```python
from build123d import *

# Parameters (mm, degrees)
SKETCH_2_W             = 85
SKETCH_2_H             = 230
EXTRUDE_1_DEPTH        = 12
CUT_EXTRUDE_2_DEPTH    = 2
HOLE_WIZARD_M5_1_D     = 4.2
HOLE_WIZARD_M4_1_D     = 3.3
HOLE_WIZARD_M6_1_D     = 5
HOLE_WIZARD_M6_1_DEPTH = 15
HOLE_WIZARD_M6_1_TIP   = 1.502151548
CHAMFER_1_SIZE         = 2


with BuildPart() as part:
    # 草图2 → 凸台-拉伸1 (new body)
    with BuildSketch(Plane.XY):
        Rectangle(SKETCH_2_W, SKETCH_2_H)
    extrude(amount=EXTRUDE_1_DEPTH)

    # 草图16 → 切除-拉伸2 (cut)
    with BuildSketch(Plane.XY.offset(12)):
        with BuildLine():
            Line((-22, 110), (22, 110))
            ThreePointArc((22, 110), (24.121320344, 109.121320344), (25, 107))
            Line((25, 107), (25, 53))
            ThreePointArc((25, 53), (24.121320344, 50.878679656), (22, 50))
            Line((22, 50), (-22, 50))
            ThreePointArc((-22, 50), (-24.121320344, 50.878679656), (-25, 53))
            Line((-25, 53), (-25, 107))
            ThreePointArc((-25, 107), (-24.121320344, 109.121320344), (-22, 110))
        make_face()
        with BuildLine():
            Line((-37.5, -115), (37.5, -115))
            Line((37.5, -115), (37.5, -48))
            ThreePointArc((37.5, -48), (36.621320344, -45.878679656), (34.5, -45))
            Line((34.5, -45), (-34.5, -45))
            ThreePointArc((-34.5, -45), (-36.621320344, -45.878679656), (-37.5, -48))
            Line((-37.5, -48), (-37.5, -115))
        make_face()
    extrude(amount=-CUT_EXTRUDE_2_DEPTH, mode=Mode.SUBTRACT)

    # M5 螺纹孔1 (through all)
    with Locations(Plane(origin=(0, 0, 0), x_dir=(-1, 0, 0), z_dir=(0, 0, -1))):
        with Locations((-17.5, -75), (17.5, -75), (17.5, -105), (-17.5, -105)):
            Hole(HOLE_WIZARD_M5_1_D / 2)

    # M4 螺纹孔1 (through all)
    with Locations(Plane.XY.offset(12)):
        with Locations((-20, 69), (20, 69), (-20, 91), (20, 91)):
            Hole(HOLE_WIZARD_M4_1_D / 2)

    # M6 螺纹孔1
    with Locations(Plane(origin=(0, 0, 0), x_dir=(-1, 0, 0), z_dir=(0, 0, -1))):
        with Locations((-35, 107.5), (-35, 69.5), (35, 69.5), (35, 107.5), (-35, 7.5), (-35, -30.5), (35, -30.5), (35, 7.5)):
            Hole(HOLE_WIZARD_M6_1_D / 2, depth=HOLE_WIZARD_M6_1_DEPTH)
            with Locations((0, 0, -(HOLE_WIZARD_M6_1_DEPTH + HOLE_WIZARD_M6_1_TIP / 2))):  # 118° drill point
                Cone(0, HOLE_WIZARD_M6_1_D / 2, HOLE_WIZARD_M6_1_TIP, mode=Mode.SUBTRACT)

    # 倒角1
    chamfer_1_edges = [part.edges().sort_by_distance(p)[0] for p in [
        (42.5, -115, 6),
        (-42.5, -115, 6),
        (-42.5, 115, 6),
        (42.5, 115, 6),
    ]]
    chamfer(chamfer_1_edges, length=CHAMFER_1_SIZE)


solid = part.part
```
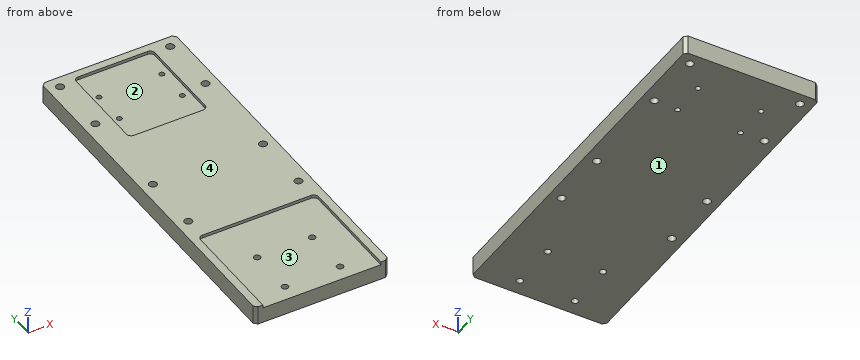
CAD build for the part. Positions are in the model's coordinates, mm. Face numbers are marked on the shaded views. A direction names the side the tool comes from. Coordinates: 2 decimals unless noted, no trailing zeros. Order: outer loops, then holes, each group sorted by start corner. A loop starts at its lowest first (then second) coordinate and runs counter-clockwise, first axis right, second up. Notation, with made-up numbers: (15.5, 23) - (38.5, 23) arc R15 ccw to (38.5, 42) - close; hole circle Ø1 at (-20.75, 0). An arc over 180 degrees is marked (long way). Answer in a Markdown table with one row per item.
1. Slice it at C-C, the plane x = -3.5. List the corners of the cut face in (y, z).
Answer:
| item | result |
|---|---|
| outline | (-115, 0) - (115, 0) - (115, 12) - (110, 12) - (110, 10) - (50, 10) - (50, 12) - (-45, 12) - (-45, 10) - (-115, 10) - close |
2. 3-axis set-ups, long thin cutter, end or side, ignore diameter. For the marked faces 3 and 4: which of +Z, -Z, +X, -X, +Y, -Y reach the whole face in a straight line?
Answer:
| item | result |
|---|---|
| face 3 | +Z, -Y |
| face 4 | +Z, +X, -X, +Y, -Y |
3. Slice it at A-A, the plane y = 7.5. List the corners of the cut face in (x, z), then the cut area to 3 significant figures.
Answer:
| item | result |
|---|---|
| outline | (-42.5, 0) - (-37.5, 0) - (-37.5, 12) - (-42.5, 12) - close; (-32.5, 0) - (32.5, 0) - (32.5, 12) - (-32.5, 12) - close; (37.5, 0) - (42.5, 0) - (42.5, 12) - (37.5, 12) - close |
| area | 900 mm² |
4. Drill centre lines: L1, parallel to Y at x = -35, z = 3.5; L2, parallel to X at y = 91, z = 5.75; L3, parallel to Y at x = 20, z = 6. Where is each one in solid material? Low to high. Write a range as from..to.
Answer:
| item | result |
|---|---|
| L1 | -115..-33, -28..5, 10..67, 72..105, 110..115 |
| L2 | -42.5..-21.65, -18.35..18.35, 21.65..42.5 |
| L3 | -115..67.35, 70.65..89.35, 92.65..115 |
5. Pull direction Y, two halves, no side cores. Call the marked faces 1 and 2: +Y half, -Y half, draft (parallel to the pull), parting line (faces both ways), or undercut.
Answer:
| item | result |
|---|---|
| face 1 | draft |
| face 2 | undercut |
6. Flat gauge pins, fed straight in: P1, Ø6.5, axis at x = -17.5, y = -75, coming from the -Z side; P2, Ø1.6, axis at x = -7.5, z = 11.5, coming from the -Y side; P3, Ø5.5, axis at x = 20, y = 91, coming from the +Z side. Where does each tip first touch, or does it go through?
Answer:
| item | result |
|---|---|
| P1 | z = 0 |
| P2 | y = -45 |
| P3 | z = 10 |
7. Slice it at D-D, the plane y = 81.5. List the corners of the cut face in (x, z), then the cut area to 3 significant figures.
Answer:
| item | result |
|---|---|
| outline | (-42.5, 0) - (42.5, 0) - (42.5, 12) - (25, 12) - (25, 10) - (-25, 10) - (-25, 12) - (-42.5, 12) - close |
| area | 920 mm² |
8. Slice it at B-B, the plane y = -105. List the corners of the cut face in (x, z).
Answer:
| item | result |
|---|---|
| outline | (-42.5, 0) - (-19.6, 0) - (-19.6, 10) - (-37.5, 10) - (-37.5, 12) - (-42.5, 12) - close; (-15.4, 0) - (15.4, 0) - (15.4, 10) - (-15.4, 10) - close; (19.6, 0) - (42.5, 0) - (42.5, 12) - (37.5, 12) - (37.5, 10) - (19.6, 10) - close |
